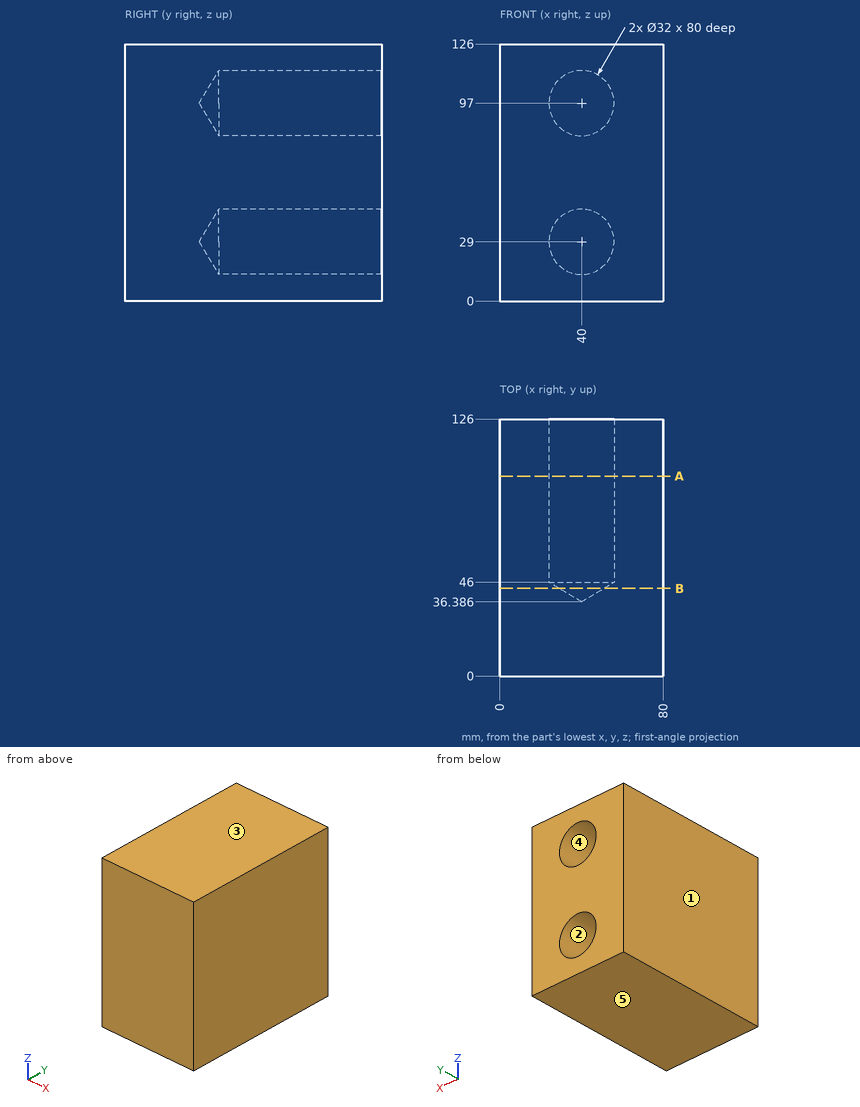
For this review, use the dimensioned drawing (mm, ordinates from the lowest corner) and the shaded views. A direction names the side the tool comes from. Give positions to 0.01 mm unless a question says otherwise; leave off trailing zeros. Loops run counter-clockwise (first coordinate to the right, second up) from the corner with the lowest first, then second, coordinate; pieces in that order, holes last.
Item 1: Take a section at A-A, the plane y = 98. State the section outline as (x, z) points.
Item 2: Draft analysis for pull direction Z (two halves, no side actions). For the marked faces 1, 2 and 3, state which applies: +Z half, -Z half, draft (parallel to the pull), parting line (faces both ways), or undercut.
Item 3: Tool access review of the marked faces 4 and 5: name each direction out of +Z, -Z, +X, -X, +Y, -Y from which nothing blocks a thin tool from reaching the whole face with its end or side.
Item 4: Insertion check: pin 1 (19 mm diameter, centred on x = 40, z = 29, fed in from +Y) (1 decimal). The pin has a flat end and moves straight along its axis. Give the tip position at first contact, or say it passes through.
Item 5: Take a section at B-B, the plane y = 43. State the section outline as (x, z) points, and give its area (3 significant figures).
Item 6: For line 1 along Z through (x, y) = (40, 105); line 2 along X through (y, z) = (69, 97); line 3 along Z through (x, y) = (43, 114.5), list the stretches that pass through material, from the lowest coordinate up.
Calculated:
1. outline: (0, 0) - (80, 0) - (80, 126) - (0, 126) - close; hole circle Ø32 at (40, 29); hole circle Ø32 at (40, 97)
2. face 1: draft
2. face 2: undercut
2. face 3: +Z half
3. face 4: +Y
3. face 5: -Z, +X, -X, +Y, -Y
4. pin 1: stops at y = 42.1
5. outline: (0, 0) - (80, 0) - (80, 126) - (0, 126) - close; hole circle Ø22.01 at (40, 29); hole circle Ø22.01 at (40, 97)
5. area: 9,320 mm2
6. line 1: z = 0 to 13, 45 to 81, 113 to 126
6. line 2: x = 0 to 24, 56 to 80
6. line 3: z = 0 to 13.28, 44.72 to 81.28, 112.72 to 126
